Build history of the part. All positions in model axes, mm. Round coordinates to 2 decimals unless told otherwise and drop trailing zeros. Loops run counter-clockwise (first coordinate to the right, second up) from the corner with the lowest first, then second, coordinate; pieces in that order, holes last. Notation, with made-up numbers: M 25,13 L 71,13 A22 cw 71,51 Z; hole C 21.25,83.25 d7. An arc over 180 degrees is marked long. One line per item, written item: value.
```python
from build123d import *

# Parameters (mm, degrees)
SKETCH1_W           = 30
SKETCH1_H           = 150
BOSS_EXTRUDE1_DEPTH = 15
CHAMFER1_SIZE       = 5
SKETCH2_R           = 5.25
CUT_EXTRUDE1_DEPTH  = 43


with BuildPart() as part:
    # Sketch1 → Boss-Extrude1 (new body)
    with BuildSketch(Plane.XY):
        Rectangle(SKETCH1_W, SKETCH1_H)
    extrude(amount=BOSS_EXTRUDE1_DEPTH)

    # Chamfer1
    chamfer1_edges = [part.edges().sort_by_distance(p)[0] for p in [
        (15, -75, 7.5),
        (-15, -75, 7.5),
        (-15, 75, 7.5),
        (15, 75, 7.5),
    ]]
    chamfer(chamfer1_edges, length=CHAMFER1_SIZE)

    # Sketch2 → Cut-Extrude1 (cut)
    with BuildSketch(Plane.XY.offset(15)):
        with Locations((0, 60)):
            Circle(SKETCH2_R)
        with Locations((0, -5)):
            Circle(SKETCH2_R)
        with Locations((0, -20)):
            Circle(SKETCH2_R)
        with Locations((0, -35)):
            Circle(SKETCH2_R)
        with Locations((0, -50)):
            Circle(SKETCH2_R)
        with Locations((0, -65)):
            Circle(SKETCH2_R)
    extrude(amount=-CUT_EXTRUDE1_DEPTH, mode=Mode.SUBTRACT)


solid = part.part
```
Item 1: Slice it at D-D, the plane y = -46. Give the cut face in (x, z), and give its area (3 significant figures).
Check values:
outline: M -15,0 L -3.4,0 L -3.4,15 L -15,15 Z; M 3.4,0 L 15,0 L 15,15 L 3.4,15 Z
area: 348 mm2
Item 2: Slice it at A-A, the plane y = -65. Give the cut face in (x, z).
Check values:
outline: M -15,0 L -5.25,0 L -5.25,15 L -15,15 Z; M 5.25,0 L 15,0 L 15,15 L 5.25,15 Z
Item 3: Drop a flat-ended pin along its axis: P1, Ø6.5, axis at x = 0, y = -35, coming from the +Z side. Give the stop position or say it passes through.
Check values:
P1: passes through
Item 4: Pull direction Y, two halves, no side cores. Call faces 1 (the face through (0, -75, 7)), 2 (the face through (5, -18.4, 7.6)), 3 (the face through (15, -1, 7)), 4 (the face through (-1.138, -70.125, 7.605)): pulls with the +Y half, pulls with the -Y half, needs draft (parallel to the pull), parting line crosses it, or undercut.
Check values:
face 1: pulls with the -Y half
face 2: undercut
face 3: needs draft
face 4: undercut
Item 5: Wall check: line 1 along X through (y, z) = (-50.5, 12.75); line 2 along X through (y, z) = (-68.5, 6.25); line 3 along Y through (x, z) = (12.75, 1). Give the ranges that are in metal, low to high.
Check values:
line 1: x = -15 to -5.23, 5.23 to 15
line 2: x = -15 to -3.91, 3.91 to 15
line 3: y = -72.25 to 72.25
Item 6: Slice it at C-C, the plane z = 5. Give the cut face in (x, y).
Check values:
outline: M -15,-70 L -10,-75 L 10,-75 L 15,-70 L 15,70 L 10,75 L -10,75 L -15,70 Z; hole C 0,-65 d10.5; hole C 0,-50 d10.5; hole C 0,-35 d10.5; hole C 0,-20 d10.5; hole C 0,-5 d10.5; hole C 0,60 d10.5
Item 7: Slice it at B-B, the plane x = 0. Give the cut face in (y, z), and give its area (4 significant figures).
Check values:
outline: M -75,0 L -70.25,0 L -70.25,15 L -75,15 Z; M -59.75,0 L -55.25,0 L -55.25,15 L -59.75,15 Z; M -44.75,0 L -40.25,0 L -40.25,15 L -44.75,15 Z; M -29.75,0 L -25.25,0 L -25.25,15 L -29.75,15 Z; M -14.75,0 L -10.25,0 L -10.25,15 L -14.75,15 Z; M 0.25,0 L 54.75,0 L 54.75,15 L 0.25,15 Z; M 65.25,0 L 75,0 L 75,15 L 65.25,15 Z
area: 1,305 mm2
